For this review, use the dimensioned drawing (mm, ordinates from the lowest corner) and the shaded views. A direction names the side the tool comes from. Coordinates: 2 decimals unless noted, no trailing zeros. Write each loop counter-clockwise with the first axis right and the second up, starting at its lowest first coordinate (ties: lowest second). Pieces come first, ordered by that corner, then holes. Notation, with made-up numbers: (-15, -11) - (27, -11) arc R22 cw to (27, 18) - close; hole circle Ø2 at (-27.5, -30.5). An arc over 180 degrees is marked (long way). Use one line per item in the form item = value. Start each with the question number.
1) For L1, parallel to X at y = 15, z = 22.5; L2, parallel to Y at x = 12, z = 75.5, list the stretches that pass through material, from the lowest coordinate up. Write a range as from..to.
2) We need section C-C (x = 57). Give the boundary of the cut face in (y, z).
3) Insertion check: P1, Ø2, axis at x = 79, z = 18, coming from the -Y side. The pin has a flat end and moves straight along its axis. Give the tip position at first contact, or say it passes through.
4) Tool access review of the marked faces 1 and 2: name each direction out of +Z, -Z, +X, -X, +Y, -Y from which nothing blocks a thin tool from reaching the whole face with its end or side.
5) We need section B-B (z = 36.5). Give the boundary of the cut face in (x, y), plus the area to 3 significant figures.
6) Mouldability with a two-part tool opening along X and no side actions: class the marked faces 3, 4 and 5 as pulls with the +X half, pulls with the -X half, needs draft (parallel to the pull), parting line crosses it, or undercut.
7) We need section A-A (y = 27.5). Give the boundary of the cut face in (x, z), plus the area to 3 significant figures.
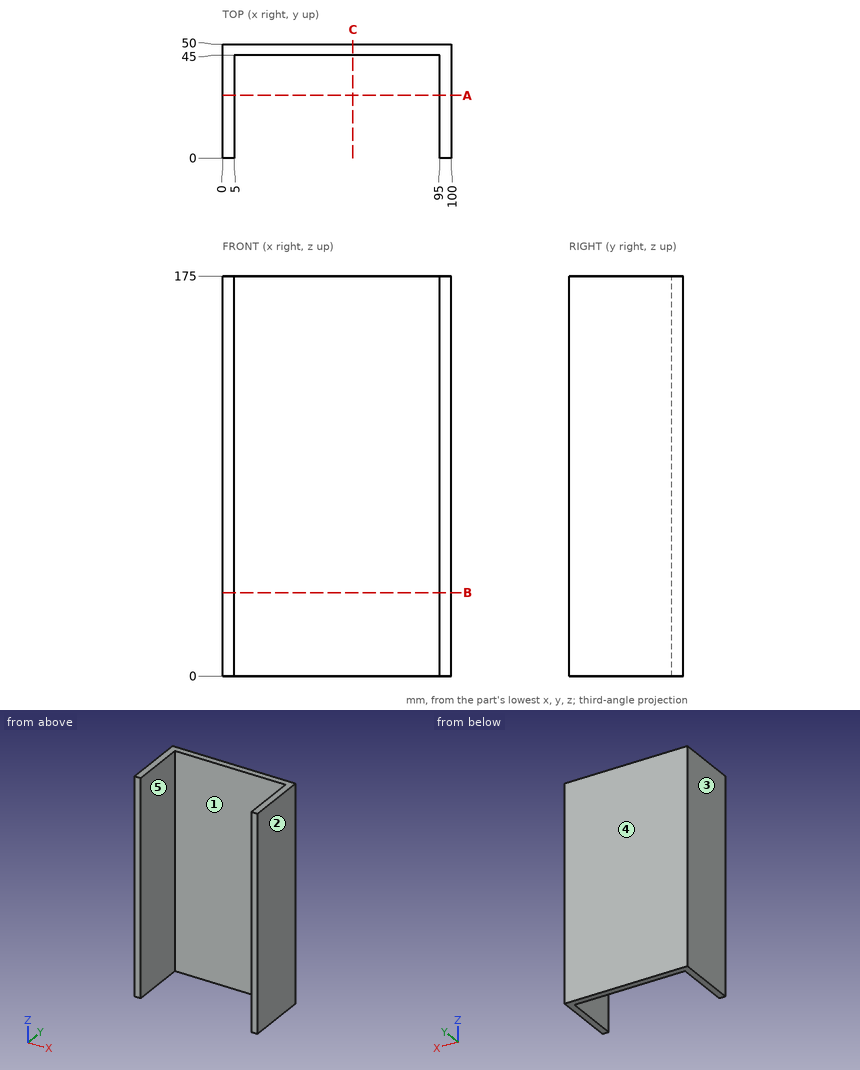
Determined:
q1.L1 = 0..5, 95..100
q1.L2 = 45..50
q2.outline = (45, 0) - (50, 0) - (50, 175) - (45, 175) - close
q3.P1 = 45
q4.face_1 = +Z, -Z, -Y
q4.face_2 = +Z, -Z, +X, +Y, -Y
q5.outline = (0, 0) - (5, 0) - (5, 45) - (95, 45) - (95, 0) - (100, 0) - (100, 50) - (0, 50) - close
q5.area = 950 mm²
q6.face_3 = pulls with the -X half
q6.face_4 = needs draft
q6.face_5 = undercut
q7.outline = (0, 0) - (5, 0) - (5, 175) - (0, 175) - close; (95, 0) - (100, 0) - (100, 175) - (95, 175) - close
q7.area = 1,750 mm²
